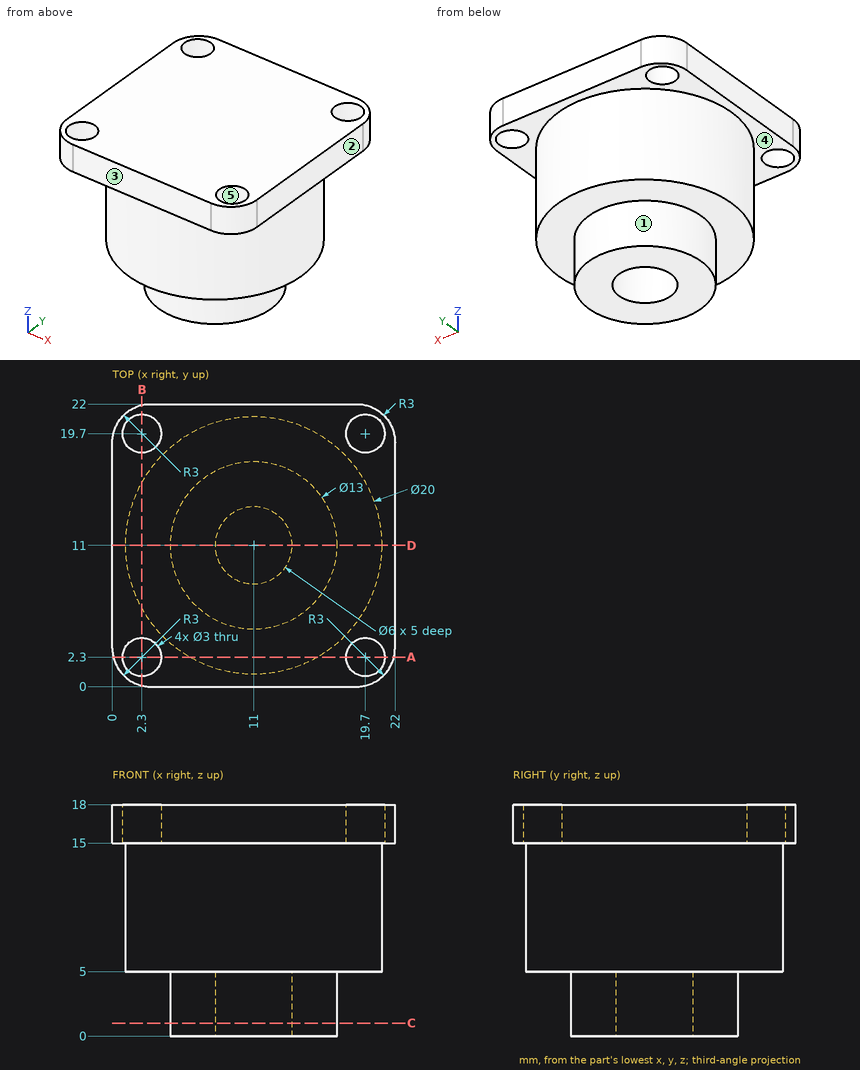
Design review of the part shown in the three views and the two pictorial views. Dimensions are in mm from the part's minimum x, y and z. A direction names the side the tool comes from. Coordinates: 2 decimals unless noted, no trailing zeros. Order: outer loops, then holes, each group sorted by start corner. A loop starts at its lowest first (then second) coordinate and runs counter-clockwise, first axis right, second up. Notation, with made-up numbers: (50, 39.5) - (107, 39.5) arc R26 cw to (107, 71.5) - close; hole circle Ø11 at (-25, 29). An arc over 180 degrees is marked (long way). Answer as CSV lines item,"result". Start each with the question number.
1) Add section D-D (y = 11). State the section outline as (x, z) points, then the cut area to 3 significant figures.
2) Machinability: for the marked faces 1 and 2, which of the approach directions +Z, -Z, +X, -X, +Y, -Y give a long, thin tool a straight path to every point of the face, cutting with its end or side? Answer none if there is none.
3) Draft analysis for pull direction Y (two halves, no side actions). For the marked faces 3, 4 and 5, state which applies: +Y half, -Y half, draft (parallel to the pull), parting line (faces both ways), or undercut.
4) Insertion check: P1, Ø1.8, axis at x = 12, y = 11.5, coming from the -Z side; P2, Ø2.5, axis at x = 2.3, y = 2.3, coming from the -Z side; P3, Ø10, axis at x = 2.5, z = 4.5, coming from the +Y side. Each pin has a flat end and moves straight along its axis. Give the tip position at first contact, or say it passes through.
5) Add section A-A (y = 2.3). State the section outline as (x, z) points.
6) Add section C-C (z = 1). State the section outline as (x, y) points, then the cut area to 3 significant figures.
7) To check wall thickness, follow line 1 along Y through (x, z) = (2.3, 15.65); line 2 along Z through (x, y) = (6, 6.75); line 3 along Z through (x, y) = (1, 15.75). State the ranges of each line that lie inside material, in increasing order. Write a range as [from, to].
Result:
1,outline,"(0, 15) - (1, 15) - (1, 5) - (4.5, 5) - (4.5, 0) - (8, 0) - (8, 5) - (14, 5) - (14, 0) - (17.5, 0) - (17.5, 5) - (21, 5) - (21, 15) - (22, 15) - (22, 18) - (0, 18) - close"
1,area,"301 mm^2"
2,face 1,"-Z"
2,face 2,"+Z, -Z, +X, +Y, -Y"
3,face 3,"-Y half"
3,face 4,"draft"
3,face 5,"undercut"
4,P1,"z = 5"
4,P2,"through"
4,P3,"y = 20.36"
5,outline,"(0.08, 15) - (0.8, 15) - (0.8, 18) - (0.08, 18) - close; (3.8, 15) - (6.07, 15) - (6.07, 5) - (15.93, 5) - (15.93, 15) - (18.2, 15) - (18.2, 18) - (3.8, 18) - close; (21.2, 15) - (21.92, 15) - (21.92, 18) - (21.2, 18) - close"
6,outline,"circle Ø13 at (11, 11); hole circle Ø6 at (11, 11)"
6,area,"104 mm^2"
7,line 1,"[0.08, 0.8], [3.8, 18.2], [21.2, 21.92]"
7,line 2,"[5, 18]"
7,line 3,"[15, 18]"
